Read the model definition and answer for the solid it produces. Units are mm, in the model's axes. A direction names the side the tool comes from. Coordinates: 2 decimals unless noted, no trailing zeros. Loops run counter-clockwise (first coordinate to the right, second up) from the corner with the lowest first, then second, coordinate; pieces in that order, holes last. Notation, with made-up numbers: (81.25, 26) -> (118.25, 26) arc R22 cw to (118.25, 36) -> close; hole circle Ø9 at (-18, 26.5). An arc over 180 degrees is marked (long way). Answer in a Markdown table with one row per item.
```python
from build123d import *

# Parameters (mm, degrees)
SKETCH1_R             = 5
BOSS_EXTRUDE1_DEPTH   = 48
SKETCH2_R             = 3
BOSS_EXTRUDE2_DEPTH   = 6.5
M4_TAPPED_HOLE1_D     = 3.3
M4_TAPPED_HOLE1_DEPTH = 10.1
M4_TAPPED_HOLE1_TIP   = 0.991420021
M5_TAPPED_HOLE1_D     = 4.2
M5_TAPPED_HOLE1_DEPTH = 12.4
M5_TAPPED_HOLE1_TIP   = 1.2618073
CHAMFER1_SIZE         = 0.5
CUT_EXTRUDE1_START    = 5
SKETCH7_W             = 10
SKETCH7_H             = 5
CUT_EXTRUDE1_DEPTH    = 1.5


with BuildPart() as part:
    # Sketch1 → Boss-Extrude1 (new body)
    with BuildSketch(Plane.XY):
        Circle(SKETCH1_R)
    extrude(amount=BOSS_EXTRUDE1_DEPTH)

    # Sketch2 → Boss-Extrude2 (add)
    with BuildSketch(Plane.XY.offset(48)):
        with Locations(Location((0, 0, 0), (0, 0, 180))):
            Circle(SKETCH2_R)
    extrude(amount=BOSS_EXTRUDE2_DEPTH)

    # M4 Tapped Hole1
    with Locations(Plane.XY.offset(54.5)):
        with Locations((0, 0)):
            Hole(M4_TAPPED_HOLE1_D / 2, depth=M4_TAPPED_HOLE1_DEPTH)
            with Locations((0, 0, -(M4_TAPPED_HOLE1_DEPTH + M4_TAPPED_HOLE1_TIP / 2))):  # 118° drill point
                Cone(0, M4_TAPPED_HOLE1_D / 2, M4_TAPPED_HOLE1_TIP, mode=Mode.SUBTRACT)

    # M5 Tapped Hole1
    with Locations(Plane(origin=(0, 0, 0), x_dir=(-1, 0, 0), z_dir=(0, 0, -1))):
        with Locations((0, 0)):
            Hole(M5_TAPPED_HOLE1_D / 2, depth=M5_TAPPED_HOLE1_DEPTH)
            with Locations((0, 0, -(M5_TAPPED_HOLE1_DEPTH + M5_TAPPED_HOLE1_TIP / 2))):  # 118° drill point
                Cone(0, M5_TAPPED_HOLE1_D / 2, M5_TAPPED_HOLE1_TIP, mode=Mode.SUBTRACT)

    # Chamfer1
    chamfer1_edges = [part.edges().sort_by_distance(p)[0] for p in [
        (-5, 0, 0),
        (-5, 0, 48),
        (3, 0, 54.5),
    ]]
    chamfer(chamfer1_edges, length=CHAMFER1_SIZE)

    # Sketch7 → Cut-Extrude1 (cut, symmetric)
    with BuildSketch(Plane(origin=(0, 0, 0), x_dir=(1, 0, 0), z_dir=(0, 1, 0)).offset(CUT_EXTRUDE1_START)):
        with Locations((0, -12.5)):
            Rectangle(SKETCH7_W, SKETCH7_H)
    cut_extrude1 = extrude(amount=CUT_EXTRUDE1_DEPTH, both=True, mode=Mode.SUBTRACT)

    # Mirror1: Cut-Extrude1 across plane
    add(cut_extrude1.mirror(Plane.ZX), mode=Mode.SUBTRACT)


solid = part.part
```
1. A cutting plane is placed at B-B on z = 50. Give the vertices of the cut face in (x, y).
A:
| item | result |
|---|---|
| outline | circle Ø6 at (0, 0); hole circle Ø3.3 at (0, 0) |
2. Given pin 1 Ø2 at (x, z) = (-1.5, 18.5) entering from +Y; pin 2 Ø3 at (y, z) = (-3, 11.5) entering from +X; pin 3 Ø1 at (y, z) = (-3.5, 8) entering from -X, each flat-ended and moving along its own axis, determine where each tip first touches the part or whether it passes through.
A:
| item | result |
|---|---|
| pin 1 | stops at y = 4.97 |
| pin 2 | stops at x = 4.77 |
| pin 3 | stops at x = -4 |
3. A tool of negligible diameter and unlimited length cuts with its end or side. For faces 4 (the flat face through (0, 3.5, 12)), 5 (the cylindrical face through (2.003, 0.631, 6.287)), 6 (the flat face through (0, -3.5, 12)), from which of +Z, -Z, +X, -X, +Y, -Y can it reach the whole face along a straight path? Write none if from no direction.
A:
| item | result |
|---|---|
| face 4 | +X, -X, +Y |
| face 5 | -Z |
| face 6 | +X, -X, -Y |
4. The mould has two halves that part along X. Classify faces 1 (the cylindrical face through (-5, 0, 24)), 2 (the cylindrical face through (1.216, 1.115, 49.379)), 3 (the flat face through (-2.1, -0.9, 0)): pulls with the +X half, pulls with the -X half, needs draft (parallel to the pull), parting line crosses it, or undercut.
A:
| item | result |
|---|---|
| face 1 | parting line crosses it |
| face 2 | undercut |
| face 3 | needs draft |
5. A cutting plane is placed at A-A on z = 33.5. Give the vertices of the cut face in (x, y).
A:
| item | result |
|---|---|
| outline | circle Ø10 at (0, 0) |
6. Find the intervals of material crossed by probe 1 along Y at (x, z) = (0, 3); probe 2 along Y at (x, z) = (0, 48.5); probe 3 along Z at (x, y) = (-1, -4), in increasing order.
A:
| item | result |
|---|---|
| probe 1 | y = -5 to -2.1, 2.1 to 5 |
| probe 2 | y = -3 to -1.65, 1.65 to 3 |
| probe 3 | z = 0 to 10, 15 to 48 |
